Input: part model. Units: mm. Frame: model coordinates. A direction names the side the tool comes from. Coordinates: 2 decimals unless noted, no trailing zeros. Write each loop counter-clockwise with the first axis right and the second up, starting at its lowest first coordinate (ties: lowest second). Pieces come first, ordered by that corner, then holes. Notation, with made-up numbers: M 72.5,32 L 120.5,32 A12 cw 120.5,44 Z; hole C 23.5,24.5 d11. An arc over 180 degrees is marked long. Use CSV: the item, a comma, the result in double quotes.
```python
from build123d import *

# Parameters (mm, degrees)
EXTRUDE_1_DEPTH = 110


with BuildPart() as part:
    # 草图1 → 凸台-拉伸1 (new, symmetric)
    with BuildSketch(Plane.XY):
        Polygon((-155, 0), (0, 0), (0, 185), (-5, 185), (-5, 5), (-155, 5), align=None)
    extrude(amount=EXTRUDE_1_DEPTH, both=True)


solid = part.part
```
1. Section A-A (z = -78). Return loops of the section in (x, y), then the cut area to 4 significant figures.
Resolved:
outline,"M -155,0 L 0,0 L 0,185 L -5,185 L -5,5 L -155,5 Z"
area,"1,675 mm^2"
2. Section B-B (x = -33). Return loops of the section in (y, z).
Resolved:
outline,"M 0,-110 L 5,-110 L 5,110 L 0,110 Z"
3. Section C-C (y = 164). Return loops of the section in (x, z).
Resolved:
outline,"M -5,-110 L 0,-110 L 0,110 L -5,110 Z"
4. Contact query for flat-ended pins moving along their axis: pin 1 Ø2 at (x, z) = (-112, 21.5) entering from +Y; pin 2 Ø4 at (y, z) = (35, 17) entering from -X; pin 3 Ø3 at (x, z) = (-88.5, 5.5) entering from -Y. Output: stop coordinate, or through.
Resolved:
pin 1,"stops at y = 5"
pin 2,"stops at x = -5"
pin 3,"stops at y = 0"
5. Material intervals for line 1 (X direction, y = 30.5, z = -3.5); line 2 (Y direction, x = -134, z = -50), sorted ascending. Write a range as [from, to].
Resolved:
line 1,"x = [-5, 0]"
line 2,"y = [0, 5]"
6. Access query for faces 1 (the flat face through (-79, 5, 2)), 2 (the flat face through (-3, 52, -110)). Directions: +Z, -Z, +X, -X, +Y, -Y. A direction counts if a zero-diameter tool reaches every point of the face in a straight line with its end or side. Return the directions, or none.
Resolved:
face 1,"+Z, -Z, -X, +Y"
face 2,"-Z, +X, -X, +Y, -Y"
